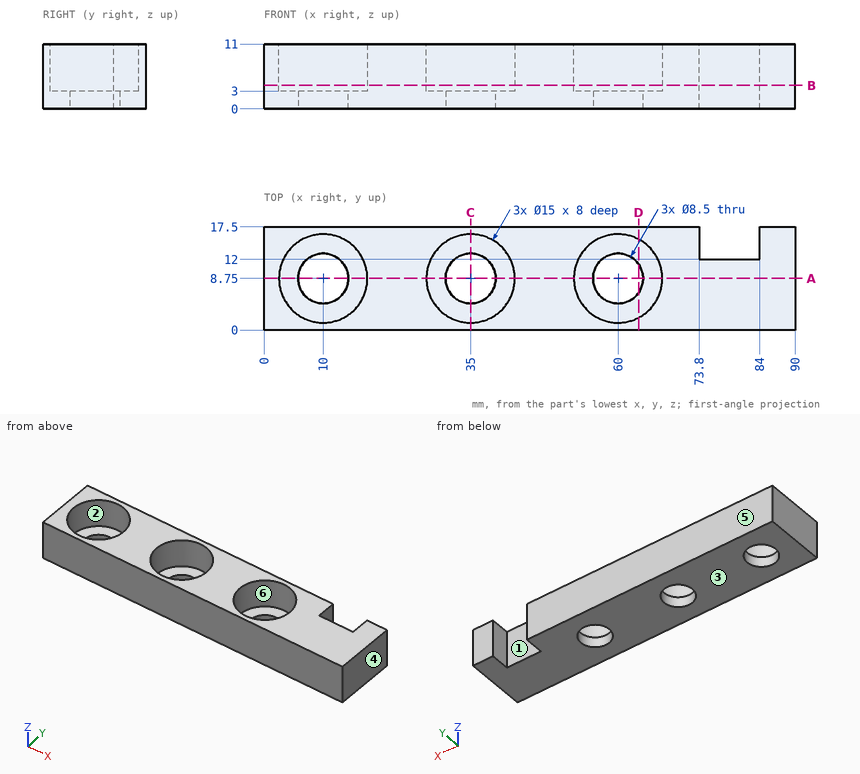
Drawing for the job (mm, zero at the part's lowest x, y, z). A direction names the side the tool comes from. Coordinates: 2 decimals unless noted, no trailing zeros. Write each loop counter-clockwise with the first axis right and the second up, starting at its lowest first coordinate (ties: lowest second). Pieces come first, ordered by that corner, then holes. Notation, with made-up numbers: (-11, 31) -> (32, 31) arc R21 ccw to (32, 66) -> close; hole circle Ø7 at (82.5, -18). An arc over 180 degrees is marked (long way). One line per item, written item: value. Start each with the question number.
1) Probe probe 1 along X at (y, z) = (8.75, 1.2); probe 2 along Y at (x, z) = (10, 1.35); probe 3 along X at (y, z) = (14.5, 9.5). List the from-to ranges inside material, lowest first.
2) Slice it at A-A on y = 8.75. Write the cut outline in (x, z), then the cut area to 4 significant figures.
3) Which spindle directions (+Z, -Z, +X, -X, +Y, -Y) get a long thin tool onto all of the face, cutting with end or side? Do the marked faces 5 and 6. Say none if no direction does.
4) Slice it at C-C on x = 35. Write the cut outline in (y, z), then the cut area to 3 significant figures.
5) Slice it at D-D on x = 63.5. Write the cut outline in (y, z), then the cut area to 3 significant figures.
6) Pull direction X, two halves, no side cores. Call the marked faces 1, 2, 3 and 4: +X half, -X half, draft (parallel to the pull), parting line (faces both ways), or undercut.
7) Slice it at B-B on z = 4. Write the cut outline in (x, y), then the cut area to 3 significant figures.
8) Flat gauge pins, fed straight in: pin 1 Ø3 at (x, z) = (78.5, 4.5) entering from +Y; pin 2 Ø7.5 at (x, y) = (33, 6.5) entering from +Z; pin 3 Ø7.5 at (x, y) = (60, 8.75) entering from +Z. Where does each tip first touch, or does it go through?
Answers follow:
1. probe 1: 0 to 5.75, 14.25 to 30.75, 39.25 to 55.75, 64.25 to 90
1. probe 2: 0 to 4.5, 13 to 17.5
1. probe 3: 0 to 5.18, 14.82 to 30.18, 39.82 to 55.18, 64.82 to 73.8, 84 to 90
2. outline: (0, 0) -> (5.75, 0) -> (5.75, 3) -> (2.5, 3) -> (2.5, 11) -> (0, 11) -> close; (14.25, 0) -> (30.75, 0) -> (30.75, 3) -> (27.5, 3) -> (27.5, 11) -> (17.5, 11) -> (17.5, 3) -> (14.25, 3) -> close; (39.25, 0) -> (55.75, 0) -> (55.75, 3) -> (52.5, 3) -> (52.5, 11) -> (42.5, 11) -> (42.5, 3) -> (39.25, 3) -> close; (64.25, 0) -> (90, 0) -> (90, 11) -> (67.5, 11) -> (67.5, 3) -> (64.25, 3) -> close
2. area: 553.5 mm2
3. face 5: +Z, -Z, +X, -X, +Y
3. face 6: +Z
4. outline: (0, 0) -> (4.5, 0) -> (4.5, 3) -> (1.25, 3) -> (1.25, 11) -> (0, 11) -> close; (13, 0) -> (17.5, 0) -> (17.5, 11) -> (16.25, 11) -> (16.25, 3) -> (13, 3) -> close
4. area: 47.0 mm2
5. outline: (0, 0) -> (6.34, 0) -> (6.34, 3) -> (2.12, 3) -> (2.12, 11) -> (0, 11) -> close; (11.16, 0) -> (17.5, 0) -> (17.5, 11) -> (15.38, 11) -> (15.38, 3) -> (11.16, 3) -> close
5. area: 71.9 mm2
6. face 1: undercut
6. face 2: undercut
6. face 3: draft
6. face 4: +X half
7. outline: (0, 0) -> (90, 0) -> (90, 17.5) -> (84, 17.5) -> (84, 12) -> (73.8, 12) -> (73.8, 17.5) -> (0, 17.5) -> close; hole circle Ø15 at (10, 8.75); hole circle Ø15 at (35, 8.75); hole circle Ø15 at (60, 8.75)
7. area: 989 mm2
8. pin 1: y = 12
8. pin 2: z = 3
8. pin 3: through
